The figure shows three views and two pictorial views of one solid part (mm, origin at its lowest corner). Answer the questions. Coordinates: 2 decimals unless noted, no trailing zeros. Loops run counter-clockwise (first coordinate to the right, second up) from the corner with the lowest first, then second, coordinate; pieces in that order, holes last. Notation, with made-up numbers: (-40, -33.75) -> (-6, -33.75) arc R23 cw to (-6, -22.75) -> close; hole circle Ø7 at (34.5, 35). An arc over 180 degrees is marked (long way). Use a Markdown table: item, result. Add a question column.
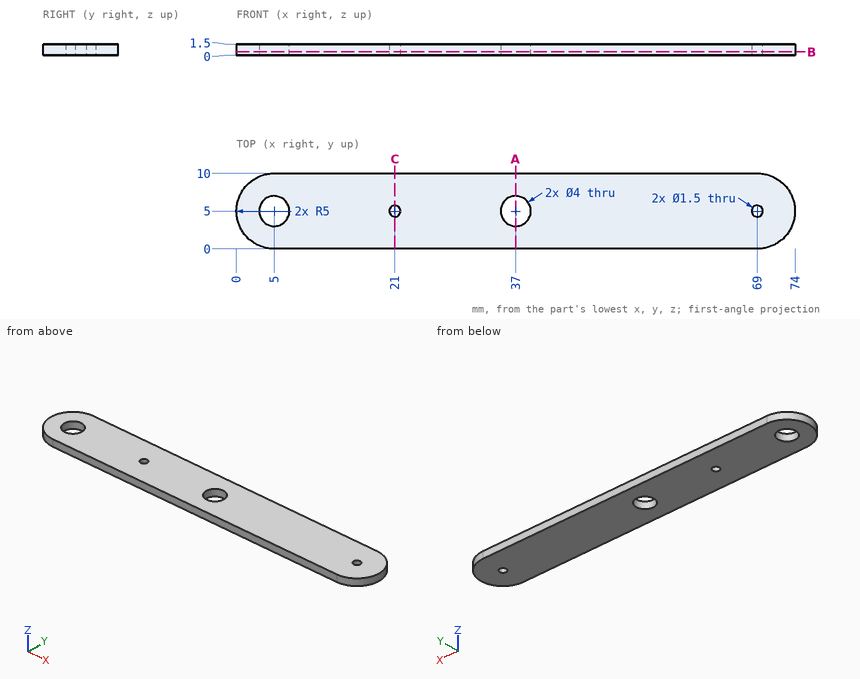
Item 1: Find the intervals of material crossed by probe 1 along Y at (x, z) = (37, 0.7); probe 2 along Y at (x, z) = (21, 1.1); probe 3 along X at (y, z) = (2.75, 0.7), in increasing order.
Item 2: Section C-C (x = 21) is taken. Determine the outline of the cut face in (y, z).
Item 3: Section A-A (x = 37) is taken. Determine the outline of the cut face in (y, z).
Item 4: Section B-B (z = 0.45) is taken. Determine the outline of the cut face in (x, y), then the cut area to 3 significant figures.
Output:
| question | item | result |
|---|---|---|
| 1 | probe 1 | y = 0 to 3, 7 to 10 |
| 1 | probe 2 | y = 0 to 4.25, 5.75 to 10 |
| 1 | probe 3 | x = 0.53 to 73.47 |
| 2 | outline | (0, 0) -> (4.25, 0) -> (4.25, 1.5) -> (0, 1.5) -> close; (5.75, 0) -> (10, 0) -> (10, 1.5) -> (5.75, 1.5) -> close |
| 3 | outline | (0, 0) -> (3, 0) -> (3, 1.5) -> (0, 1.5) -> close; (7, 0) -> (10, 0) -> (10, 1.5) -> (7, 1.5) -> close |
| 4 | outline | (5, 0) -> (69, 0) arc R5 ccw to (69, 10) -> (5, 10) arc R5 ccw to start; hole circle Ø4 at (5, 5); hole circle Ø1.5 at (21, 5); hole circle Ø4 at (37, 5); hole circle Ø1.5 at (69, 5) |
| 4 | area | 690 mm2 |
